Source: CAD feature listing. Evaluate the final solid. Frame: model axes, mm. A direction names the side the tool comes from. Coordinates: 2 decimals unless noted, no trailing zeros. Loops run counter-clockwise (first coordinate to the right, second up) from the corner with the lowest first, then second, coordinate; pieces in that order, holes last.
```python
from build123d import *

# Parameters (mm, degrees)
SKETCH1_R              = 25
BOSS_EXTRUDE1_DEPTH    = 600
CHAMFER1_SIZE          = 5
M16_TAPPED_HOLE1_D     = 14
M16_TAPPED_HOLE1_DEPTH = 38
M16_TAPPED_HOLE1_TIP   = 4.206024333
M16_TAPPED_HOLE2_D     = 14
M16_TAPPED_HOLE2_DEPTH = 38
M16_TAPPED_HOLE2_TIP   = 4.206024333


with BuildPart() as part:
    # Sketch1 → Boss-Extrude1 (new body)
    with BuildSketch(Plane(origin=(0, 0, 0), x_dir=(1, 0, 0), z_dir=(0, 1, 0))):
        with Locations(Location((0, 0, 0), (0, 0, 270))):
            Circle(SKETCH1_R)
    extrude(amount=BOSS_EXTRUDE1_DEPTH)

    # Chamfer1
    chamfer1_edges = [part.edges().sort_by_distance(p)[0] for p in [
        (0, 0, -25),
        (0, 600, -25),
    ]]
    chamfer(chamfer1_edges, length=CHAMFER1_SIZE)

    # M16 Tapped Hole1
    with Locations(Plane(origin=(0, 600, 0), x_dir=(1, 0, 0), z_dir=(0, 1, 0))):
        with Locations((0, 0)):
            Hole(M16_TAPPED_HOLE1_D / 2, depth=M16_TAPPED_HOLE1_DEPTH)
            with Locations((0, 0, -(M16_TAPPED_HOLE1_DEPTH + M16_TAPPED_HOLE1_TIP / 2))):  # 118° drill point
                Cone(0, M16_TAPPED_HOLE1_D / 2, M16_TAPPED_HOLE1_TIP, mode=Mode.SUBTRACT)

    # M16 Tapped Hole2
    with Locations(Plane(origin=(0, 0, 0), x_dir=(-1, 0, 0), z_dir=(0, -1, 0))):
        with Locations((0, 0)):
            Hole(M16_TAPPED_HOLE2_D / 2, depth=M16_TAPPED_HOLE2_DEPTH)
            with Locations((0, 0, -(M16_TAPPED_HOLE2_DEPTH + M16_TAPPED_HOLE2_TIP / 2))):  # 118° drill point
                Cone(0, M16_TAPPED_HOLE2_D / 2, M16_TAPPED_HOLE2_TIP, mode=Mode.SUBTRACT)


solid = part.part
```
Q1. Section query A-A on y = 163. Return the cut outline in (x, z).
Q2. First-contact query: pin 1 Ø2 at (x, y) = (16.5, 203) entering from +Z; pin 2 Ø12 at (y, z) = (520.5, 19) entering from -X; pin 3 Ø6 at (x, z) = (-17.5, -16.5) entering from +Y; pin 4 Ø2 at (x, z) = (-7, -1.5) entering from -Y. Flat tips, straight axial feed; report the tip coordinate or a pass-through.
Q3. Material intervals for line 1 along X through (y, z) = (158.5, 0); line 2 along Z through (x, y) = (15, 134); line 3 along Z through (x, y) = (-1, 167), sorted ascending.
Q4. Reachability of faces 1 (the cylindrical face through (-6.466, 580.734, 2.681)), 2 (the flat face through (0, 600, 9)), 3 (the cylindrical face through (6.466, 19.266, 2.681)) from +Z, -Z, +X, -X, +Y, -Y: full face, straight path, thin tool, end or side. Return the list, or none.
Q5. Draft query along X for faces 4 (the flat face through (0, 0, 9)), 5 (the conical face through (-0.264, 558.524, 1.187)), 6 (the cylindrical face through (7.509, 295.87, 23.846)), 7 (the conical face through (0.264, 41.476, 1.187)). Return one class per face: released by +X, released by -X, zero draft, split by the parting line, or undercut.
Resolved:
1. outline: circle Ø50 at (0, 0)
2. pin 1: stops at z = 19.62
2. pin 2: stops at x = -21.35
2. pin 3: stops at y = 598.95
2. pin 4: stops at y = 0
3. line 1: x = -25 to 25
3. line 2: z = -20 to 20
3. line 3: z = -24.98 to 24.98
4. face 1: +Y
4. face 2: +Z, -Z, +X, -X, +Y
4. face 3: -Y
5. face 4: zero draft
5. face 5: undercut
5. face 6: split by the parting line
5. face 7: undercut
